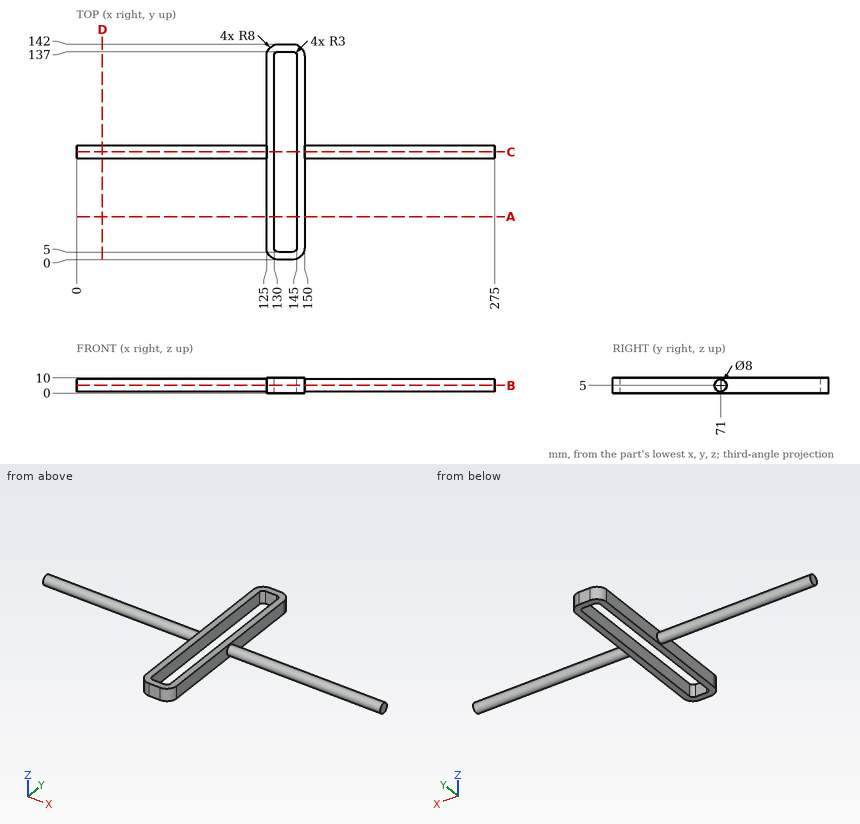
Geometry check sheet. Reference: drawing and pictorial views, mm from the part's lowest x, y, z. Coordinates: 2 decimals unless noted, no trailing zeros. Order: outer loops, then holes, each group sorted by start corner. A loop starts at its lowest first (then second) coordinate and runs counter-clockwise, first axis right, second up. Notation, with made-up numbers: (-27, -13) -> (19, -13) arc R16 ccw to (19, -9) -> close; hole circle Ø2 at (5.25, 55). An arc over 180 degrees is marked (long way). Write item = value, one per line. Start each with the question number.
1) Cross-section at A-A (y = 28.5). Enter the section's corners in (x, z).
2) Go/stop test with flat-tipped pins: P1, Ø2, axis at x = 143, y = 125.5, coming from the -Z side; P2, Ø1.5, axis at x = 100.5, z = 2, coming from the -Y side; P3, Ø1.5, axis at y = 89, z = 6.5, coming from the -X side; P4, Ø5, axis at x = 201.5, z = 2.5, coming from the -Y side. Record where each tip stops, or that it passes through.
3) Cross-section at C-C (y = 71). Enter the section's corners in (x, z), then the cut area to 3 significant figures.
4) Cross-section at B-B (z = 5). Enter the section's corners in (x, y).
5) Cross-section at D-D (x = 17). Enter the section's corners in (y, z).
6) Material ranges on L1, parallel to X at y = 24, z = 7.25; L2, parallel to Z at x = 165, y = 71; L3, parallel to Y at x = 194, z = 4.5, recorded low to high.
Ans:
q1.outline = (125, 0) -> (130, 0) -> (130, 10) -> (125, 10) -> close; (145, 0) -> (150, 0) -> (150, 10) -> (145, 10) -> close
q2.P1 = through
q2.P2 = 67.69
q2.P3 = 125
q2.P4 = 67
q3.outline = (0, 1) -> (125, 1) -> (125, 0) -> (130, 0) -> (130, 10) -> (125, 10) -> (125, 9) -> (0, 9) -> close; (145, 0) -> (150, 0) -> (150, 1) -> (275, 1) -> (275, 9) -> (150, 9) -> (150, 10) -> (145, 10) -> close
q3.area = 2,100 mm²
q4.outline = (0, 67) -> (125, 67) -> (125, 8) arc R8 ccw to (133, 0) -> (142, 0) arc R8 ccw to (150, 8) -> (150, 67) -> (275, 67) -> (275, 75) -> (150, 75) -> (150, 134) arc R8 ccw to (142, 142) -> (133, 142) arc R8 ccw to (125, 134) -> (125, 75) -> (0, 75) -> close; hole (130, 8) arc R3 ccw to (133, 5) -> (142, 5) arc R3 ccw to (145, 8) -> (145, 134) arc R3 ccw to (142, 137) -> (133, 137) arc R3 ccw to (130, 134) -> close
q5.outline = circle Ø8 at (71, 5)
q6.L1 = 125 to 130, 145 to 150
q6.L2 = 1 to 9
q6.L3 = 67.03 to 74.97
